Input: part model. Units: mm. Frame: model coordinates. A direction names the side the tool comes from. Coordinates: 2 decimals unless noted, no trailing zeros. Order: outer loops, then holes, each group sorted by start corner. A loop starts at its lowest first (then second) coordinate and runs counter-clockwise, first axis right, second up. Notation, with made-up numbers: (17, 87.25) -> (61, 87.25) arc R8 ccw to (61, 94.25) -> close; hole circle Ø7 at (58.25, 20.25). An arc over 180 degrees is marked (long way). One line per item, written item: value. Start each with the question number.
from build123d import *

# Parameters (mm, degrees)
SWEEP1_PROFILE_R = 2.5


with BuildPart() as part:
    # Sweep1: sweep along a path in Sketch1
    with BuildLine(Plane(origin=(0, 0, 0), x_dir=(1, 0, 0), z_dir=(0, 1, 0))) as sweep1_path:
        Line((0, -10), (0, -5))
        ThreePointArc((0, -5), (1.464466094, -1.464466094), (5, 0))
        Line((5, 0), (95, 0))
        ThreePointArc((95, 0), (98.535533906, -1.464466094), (100, -5))
        Line((100, -5), (100, -10))
    # Sweep1 profile (on start of the path) → Sweep1 (sweep)
    with BuildSketch(Plane(origin=(0, 0, 10), x_dir=(-1, 0, 0), z_dir=(0, 0, -1))):
        Circle(SWEEP1_PROFILE_R)
    sweep(path=sweep1_path.line)


solid = part.part
1) Mould query, pull axis X, two halves, no side actions, for faces 4 (the flat face through (100, 0, 10)), 5 (the cylindrical face through (102.385, 0.751, 7.535)). Classes: +X half, -X half, draft (parallel to the pull), parting line (faces both ways), or undercut.
2) Access query for faces 1 (the cylindrical face through (50.63, -2.44, 0.54)), 2 (the cylindrical face through (0.54, -2.44, 7.46)), 3 (the flat face through (0, 0, 10)). Directions: +Z, -Z, +X, -X, +Y, -Y. A direction counts if a zero-diameter tool reaches every point of the face in a straight line with its end or side. Return the directions, or none.
3) Section query A-A, the plane y = 0. Return the cut outline in (x, z).
4) Pin query (flat end, axial travel): pin 1 Ø2 at (x, y) = (15, 0) entering from +Z; pin 2 Ø1 at (x, y) = (25.5, -2) entering from +Z; pin 3 Ø1.5 at (y, z) = (-2, 3.5) entering from -X. Return the tip coordinate at first contact, or that it passes through.
5) Section query C-C, the plane x = 55. Return the cut outline in (y, z), plus the area to 3 significant figures.
6) Ray query, line 1 along X through (y, z) = (-0.2, 7.5); line 2 along Z through (x, y) = (20, 0.3); line 3 along X through (y, z) = (-1.3, 8.5). Return the intervals inside material, ascending. Write a range as from..to.
7) Section query B-B, the plane z = 6.5. Return the cut outline in (x, y).
Entries:
1. face 4: draft
1. face 5: undercut
2. face 1: none
2. face 2: +Z
2. face 3: +Z, +X, -X, +Y, -Y
3. outline: (-2.5, 5) arc R7.5 ccw to (5, -2.5) -> (95, -2.5) arc R7.5 ccw to (102.5, 5) -> (102.5, 10) -> (97.5, 10) -> (97.5, 5) arc R2.5 cw to (95, 2.5) -> (5, 2.5) arc R2.5 cw to (2.5, 5) -> (2.5, 10) -> (-2.5, 10) -> close
4. pin 1: stops at z = 2.5
4. pin 2: stops at z = 2
4. pin 3: stops at x = -2.03
5. outline: circle Ø5 at (0, 0)
5. area: 19.6 mm2
6. line 1: x = -2.49..2.49, 97.51..102.49
6. line 2: z = -2.48..2.48
6. line 3: x = -2.14..2.14, 97.86..102.14
7. outline: circle Ø5 at (0, 0); circle Ø5 at (100, 0)
